Drawing for the job (mm, zero at the part's lowest x, y, z). A direction names the side the tool comes from. Coordinates: 2 decimals unless noted, no trailing zeros. Write each loop counter-clockwise with the first axis right and the second up, starting at its lowest first coordinate (ties: lowest second). Pieces come first, ordered by that corner, then holes. Notation, with made-up numbers: (32.25, -4) - (47.25, -4) arc R28 ccw to (47.25, 18) - close; hole circle Ø10 at (32.5, 85.5). An arc over 180 degrees is marked (long way). Write each question's results on one line, items separated by ' | '.
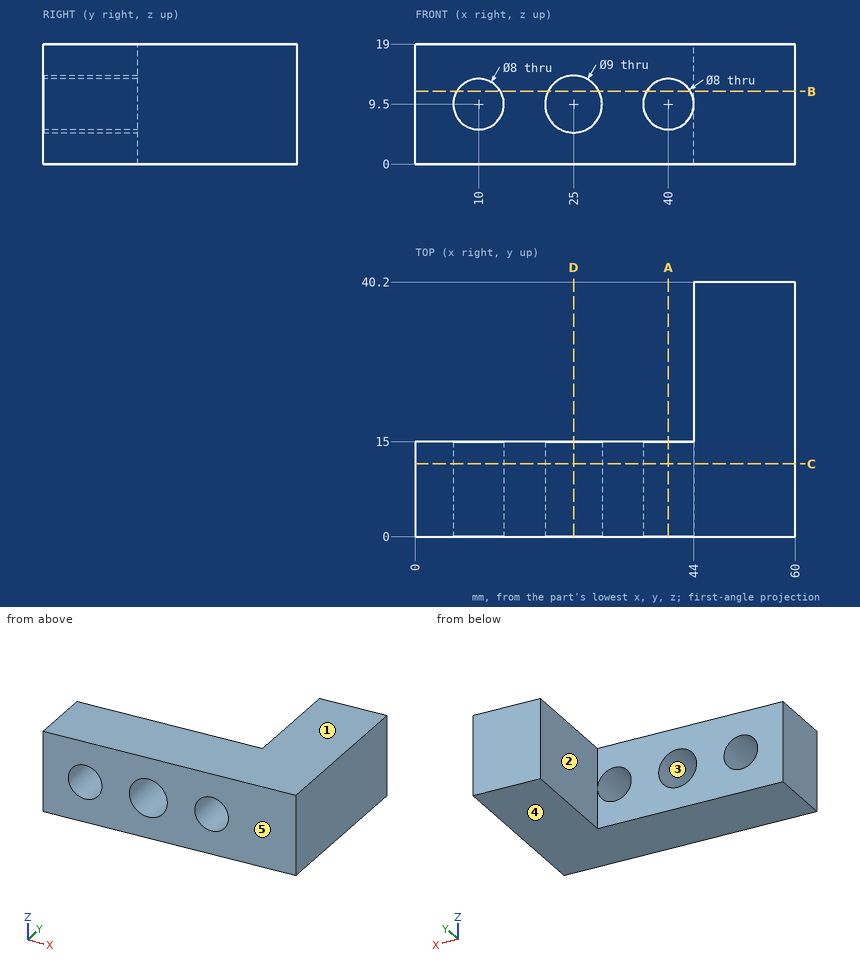
(1) Two-plate mould, pull along Z, no slides. Class the marked faces 3, 4 and 5: released by +Z, released by -Z, zero draft, split by the parting line, or undercut.
Return value:
face 3: undercut | face 4: released by -Z | face 5: zero draft
(2) Saw through at A-A on x = 40. Write the cut outline in (y, z), then the cut area to 3 significant figures.
Return value:
outline: (0, 0) - (15, 0) - (15, 5.5) - (0, 5.5) - close; (0, 13.5) - (15, 13.5) - (15, 19) - (0, 19) - close | area: 165 mm^2
(3) Saw through at C-C on y = 11.5. Write the cut outline in (x, z).
Return value:
outline: (0, 0) - (60, 0) - (60, 19) - (0, 19) - close; hole circle Ø8 at (10, 9.5); hole circle Ø9 at (25, 9.5); hole circle Ø8 at (40, 9.5)
(4) Wall check: line 1 (X direction, y = 12, z = 9.5); line 2 (Z direction, x = 40, y = 5); line 3 (Y direction, x = 23, z = 13.75). Give the ranges that are in metal, low to high. Write a range as from..to.
Return value:
line 1: x = 0..6, 14..20.5, 29.5..36, 44..60 | line 2: z = 0..5.5, 13.5..19 | line 3: y = 0..15
(5) Saw through at D-D on x = 25. Write the cut outline in (y, z), then the cut area to 3 significant figures.
Return value:
outline: (0, 0) - (15, 0) - (15, 5) - (0, 5) - close; (0, 14) - (15, 14) - (15, 19) - (0, 19) - close | area: 150 mm^2
(6) Flat gauge pins, fed straight in: P1, Ø2, axis at x = 38.5, z = 8, coming from the +Y side; P2, Ø5, axis at x = 35, z = 10.5, coming from the +Y side; P3, Ø9.5, axis at y = 28.5, z = 7, coming from the -X side. Where does each tip first touch, or does it go through?
Return value:
P1: passes through | P2: stops at y = 15 | P3: stops at x = 44
(7) 3-axis set-ups, long thin cutter, end or side, ignore diameter. For the marked faces 1 and 2: which of +Z, -Z, +X, -X, +Y, -Y reach the whole face in a straight line?
Return value:
face 1: +Z, +X, -X, +Y, -Y | face 2: +Z, -Z, -X, +Y
(8) Saw through at B-B on z = 11.5. Write the cut outline in (x, y).
Return value:
outline: (0, 0) - (6.54, 0) - (6.54, 15) - (0, 15) - close; (13.46, 0) - (20.97, 0) - (20.97, 15) - (13.46, 15) - close; (29.03, 0) - (36.54, 0) - (36.54, 15) - (29.03, 15) - close; (43.46, 0) - (60, 0) - (60, 40.2) - (44, 40.2) - (44, 15) - (43.46, 15) - close
